```python
from build123d import *

# Parameters (mm, degrees)
EXTRUDE_THIN1_DEPTH = 200
BOSS_EXTRUDE1_DEPTH = 37


with BuildPart() as part:
    # Sketch1 → Extrude-Thin1 (new body)
    with BuildSketch(Plane.XY):
        Polygon((78, 32), (83.5, 37.5), (83.5, 41.207106781), (72.707106781, 52), (-72.707106781, 52), (-83.5, 41.207106781), (-83.5, 37.5), (-78, 32), (-80.828427125, 29.171572875), (-87.5, 35.843145751), (-87.5, 42.863961031), (-74.363961031, 56), (74.363961031, 56), (87.5, 42.863961031), (87.5, 35.843145751), (80.828427125, 29.171572875), align=None)
    extrude(amount=-EXTRUDE_THIN1_DEPTH)

    # Sketch2 → Boss-Extrude1 (add)
    with BuildSketch(Plane.XY):
        Polygon((-7.989949494, 52), (3, 52), (3, 41.010050506), align=None)
    extrude(amount=-BOSS_EXTRUDE1_DEPTH)


solid = part.part
```
The model under review builds one solid part; all positions refer to its coordinate system, in mm. A direction names the side the tool comes from. Round coordinates to 2 decimals unless told otherwise and drop trailing zeros. Loops run counter-clockwise (first coordinate to the right, second up) from the corner with the lowest first, then second, coordinate; pieces in that order, holes last. Notation, with made-up numbers: M 66.25,75.5 L 87.25,75.5 A32 cw 87.25,108.5 Z; hole C -29,-5.75 d1. An arc over 180 degrees is marked long. Write item = value, one per line.
Item 1: Take a section at C-C on x = -57.5. Write out the cut boundary in (y, z).
Return value:
outline = M 52,-200 L 56,-200 L 56,0 L 52,0 Z
Item 2: Take a section at A-A on y = 47. Write out the cut boundary in (x, z).
Return value:
outline = M -83.36,-200 L -77.71,-200 L -77.71,0 L -83.36,0 Z; M -2.99,-37 L 3,-37 L 3,0 L -2.99,0 Z; M 77.71,-200 L 83.36,-200 L 83.36,0 L 77.71,0 Z
Item 3: Machinability: for faces 1 (the flat face through (-81, 35, -99)), 2 (the flat face through (-1, 48, -37)), 3 (the flat face through (-2.42, 46.43, -18.24)), which of the approach directions +Z, -Z, +X, -X, +Y, -Y give a long, thin tool a straight path to every point of the face, cutting with its end or side? Answer none if there is none.
Return value:
face_1 = +Z, -Z
face_2 = -Z, -Y
face_3 = +Z, -Z, -Y
Item 4: The part is to be moulded in two halves that separate along X. For faces 4 (the flat face through (81, 35, -99)), 5 (the flat face through (-87.5, 39, -99)), 6 (the flat face through (0, 54, -200)), say which applies: released by +X, released by -X, zero draft, split by the parting line, or undercut.
Return value:
face_4 = undercut
face_5 = released by -X
face_6 = zero draft
Item 5: Take a section at B-B on z = -44.5. Write out the cut boundary in (x, y).
Return value:
outline = M -87.5,35.84 L -80.83,29.17 L -78,32 L -83.5,37.5 L -83.5,41.21 L -72.71,52 L 72.71,52 L 83.5,41.21 L 83.5,37.5 L 78,32 L 80.83,29.17 L 87.5,35.84 L 87.5,42.86 L 74.36,56 L -74.36,56 L -87.5,42.86 Z
Item 6: Take a section at D-D on x = -5. Write out the cut boundary in (y, z), then the cut area to 3 significant figures.
Return value:
outline = M 49.01,-37 L 52,-37 L 52,-200 L 56,-200 L 56,0 L 49.01,0 Z
area = 911 mm2
Item 7: Insertion check: P1, Ø9, axis at x = -4.5, y = 45.5, coming from the -Z side; P2, Ø8, axis at x = 66.5, y = 45, coming from the +Z side; P3, Ø8, axis at y = 50.5, z = -96, coming from the -X side; P4, Ø2, axis at y = 51.5, z = -44, coming from the +X side. Each pin has a flat end and moves straight along its axis. Give the tip position at first contact, or say it passes through.
Return value:
P1 = -37
P2 = through
P3 = -83.86
P4 = 79.86
Item 8: For line 1 (X direction, y = 38, z = -143.5); line 2 (Y direction, x = -34, z = -21); line 3 (X direction, y = 44.5, z = -42), list the stretches that pass through material, from the lowest coordinate up. Write a range as [from, to].
Return value:
line_1 = [-87.5, -83.5], [83.5, 87.5]
line_2 = [52, 56]
line_3 = [-85.86, -80.21], [80.21, 85.86]
